Work out the finished part from the listing and answer in its coordinate system (mm). Give positions to 0.01 mm unless a question says otherwise; leave off trailing zeros. Order: outer loops, then holes, each group sorted by start corner. A loop starts at its lowest first (then second) coordinate and runs counter-clockwise, first axis right, second up.
```python
from build123d import *

# Parameters (mm, degrees)
SKETCH1_R                  = 4.5
BOSS_EXTRUDE1_DEPTH        = 8
M10X1_0_TAPPED_HOLE1_D     = 9
M10X1_0_TAPPED_HOLE1_DEPTH = 23
M10X1_0_TAPPED_HOLE1_TIP   = 2.703872786


with BuildPart() as part:
    # Sketch1 → Boss-Extrude1 (new body)
    with BuildSketch(Plane.XY):
        with BuildLine():
            Line((5, 20), (85, 20))
            ThreePointArc((85, 20), (88.535533906, 18.535533906), (90, 15))
            Line((90, 15), (90, -85))
            ThreePointArc((90, -85), (88.535533906, -88.535533906), (85, -90))
            Line((85, -90), (5, -90))
            ThreePointArc((5, -90), (1.464466094, -88.535533906), (0, -85))
            Line((0, -85), (0, 15))
            ThreePointArc((0, 15), (1.464466094, 18.535533906), (5, 20))
        make_face()
        with Locations((10, 10)):
            Circle(SKETCH1_R, mode=Mode.SUBTRACT)
        with Locations((80, 10)):
            Circle(SKETCH1_R, mode=Mode.SUBTRACT)
        with Locations((10, -80)):
            Circle(SKETCH1_R, mode=Mode.SUBTRACT)
        with Locations((80, -80)):
            Circle(SKETCH1_R, mode=Mode.SUBTRACT)
    extrude(amount=BOSS_EXTRUDE1_DEPTH)

    # M10x1.0 Tapped Hole1
    with Locations(Plane(origin=(45, -35, 8), x_dir=(1, 0, 0), z_dir=(0, 0, 1))):
        with Locations((0, 0)):
            Hole(M10X1_0_TAPPED_HOLE1_D / 2, depth=M10X1_0_TAPPED_HOLE1_DEPTH)
            with Locations((0, 0, -(M10X1_0_TAPPED_HOLE1_DEPTH + M10X1_0_TAPPED_HOLE1_TIP / 2))):  # 118° drill point
                Cone(0, M10X1_0_TAPPED_HOLE1_D / 2, M10X1_0_TAPPED_HOLE1_TIP, mode=Mode.SUBTRACT)


solid = part.part
```
1. The mould has two halves that part along X. Classify faces 1 (the face through (75.504, 10.198, 3.944)), 2 (the face through (90, -34, 4)), 3 (the face through (56, -34, 8)), 4 (the face through (2, -89, 4)): pulls with the +X half, pulls with the -X half, needs draft (parallel to the pull), parting line crosses it, or undercut.
Findings below:
face 1: undercut
face 2: pulls with the +X half
face 3: needs draft
face 4: pulls with the -X half
2. Straight lines are drawn through the part: probe 1 along X at (y, z) = (9.5, 2.5); probe 2 along Y at (x, z) = (80, 3); probe 3 along X at (y, z) = (7, 3.5). For each, find the intervals that lie inside material, in ascending order.
Findings below:
probe 1: x = 0 to 5.53, 14.47 to 75.53, 84.47 to 90
probe 2: y = -90 to -84.5, -75.5 to 5.5, 14.5 to 20
probe 3: x = 0 to 6.65, 13.35 to 76.65, 83.35 to 90
3. Given P1, Ø8, axis at x = 45, y = -35, coming from the -Z side, flat-ended and moving along its own axis, determine where the tip first touches the part or whether it passes through.
Findings below:
P1: passes through
4. The part is cut by section D-D (x = 80). Write down the section's boundary in (y, z), then the cut area to 3 significant figures.
Findings below:
outline: (-90, 0) - (-84.5, 0) - (-84.5, 8) - (-90, 8) - close; (-75.5, 0) - (5.5, 0) - (5.5, 8) - (-75.5, 8) - close; (14.5, 0) - (20, 0) - (20, 8) - (14.5, 8) - close
area: 736 mm2
5. The part is cut by section B-B (x = 45). Write down the section's boundary in (y, z).
Findings below:
outline: (-90, 0) - (-39.5, 0) - (-39.5, 8) - (-90, 8) - close; (-30.5, 0) - (20, 0) - (20, 8) - (-30.5, 8) - close
6. The part is cut by section A-A (y = -35). Write down the section's boundary in (x, z).
Findings below:
outline: (0, 0) - (40.5, 0) - (40.5, 8) - (0, 8) - close; (49.5, 0) - (90, 0) - (90, 8) - (49.5, 8) - close
7. The part is cut by section C-C (y = 10). Write down the section's boundary in (x, z).
Findings below:
outline: (0, 0) - (5.5, 0) - (5.5, 8) - (0, 8) - close; (14.5, 0) - (75.5, 0) - (75.5, 8) - (14.5, 8) - close; (84.5, 0) - (90, 0) - (90, 8) - (84.5, 8) - close
